```python
from build123d import *

# Parameters (mm, degrees)
BOSS_EXTRUDE1_DEPTH = 1
SKETCH2_W           = 1
SKETCH2_H           = 8.697838108
BOSS_EXTRUDE2_DEPTH = 6
SKETCH3_W           = 3.625858974
SKETCH3_H           = 24.597729298
SKETCH3_R           = 1
BOSS_EXTRUDE3_DEPTH = 1


with BuildPart() as part:
    # Sketch1 → Boss-Extrude1 (new body)
    with BuildSketch(Plane.XY):
        with BuildLine():
            Line((117.275298476, 4.348919054), (20.445206114, 4.348919054))
            ThreePointArc((20.445206114, 4.348919054), (0, 20.902620649), (-20.445206114, 4.348919054))
            Line((-20.445206114, 4.348919054), (-117.275298476, 4.348919054))
            Line((-117.275298476, 4.348919054), (-117.275298476, -4.348919054))
            Line((-117.275298476, -4.348919054), (-20.445206114, -4.348919054))
            ThreePointArc((-20.445206114, -4.348919054), (-16.73157253, -12.528927754), (-9.927442271, -18.394712283))
            Line((-9.927442271, -18.394712283), (-9.927442271, -11.244816137))
            ThreePointArc((-9.927442271, -11.244816137), (-13.314654662, -6.907964333), (-14.909922164, -1.641408252))
            Line((-14.909922164, -1.641408252), (-19.244314933, -1.641408252))
            Line((-19.244314933, -1.641408252), (-19.244314933, 1.641408252))
            Line((-19.244314933, 1.641408252), (-14.909922164, 1.641408252))
            ThreePointArc((-14.909922164, 1.641408252), (0, 15), (14.909922164, 1.641408252))
            Line((14.909922164, 1.641408252), (19.244314933, 1.641408252))
            Line((19.244314933, 1.641408252), (19.244314933, -1.641408252))
            Line((19.244314933, -1.641408252), (14.909922164, -1.641408252))
            ThreePointArc((14.909922164, -1.641408252), (13.314654662, -6.907964333), (9.927442271, -11.244816137))
            Line((9.927442271, -11.244816137), (9.927442271, -18.394712283))
            ThreePointArc((9.927442271, -18.394712283), (16.73157253, -12.528927754), (20.445206114, -4.348919054))
            Line((20.445206114, -4.348919054), (117.275298476, -4.348919054))
            Line((117.275298476, -4.348919054), (117.275298476, 4.348919054))
        make_face()
    extrude(amount=-BOSS_EXTRUDE1_DEPTH)

    # Sketch2 → Boss-Extrude2 (add)
    with BuildSketch(Plane.XY):
        with Locations((-116.775298476, 0)):
            Rectangle(SKETCH2_W, SKETCH2_H)
        with Locations((116.775298476, 0)):
            Rectangle(SKETCH2_W, SKETCH2_H)
    extrude(amount=-BOSS_EXTRUDE2_DEPTH)

    # Sketch3 → Boss-Extrude3 (add)
    # profile 1 of 2: a face of its own
    with BuildSketch(Plane.XY.offset(-6)):
        with Locations((-116.275298476, 0)):
            Rectangle(SKETCH3_W, SKETCH3_H)
        with Locations((-116.275298476, -10)):
            Circle(SKETCH3_R, mode=Mode.SUBTRACT)
        with Locations((-116.275298476, 10)):
            Circle(SKETCH3_R, mode=Mode.SUBTRACT)
    # profile 2 of 2: a face of its own
    with BuildSketch(Plane.XY.offset(-6)):
        with Locations((116.275298476, 0)):
            Rectangle(SKETCH3_W, SKETCH3_H)
        with Locations(Location((116.275298476, 10, 0), (0, 0, 180))):
            Circle(SKETCH3_R, mode=Mode.SUBTRACT)
        with Locations(Location((116.275298476, -10, 0), (0, 0, 180))):
            Circle(SKETCH3_R, mode=Mode.SUBTRACT)
    extrude(amount=BOSS_EXTRUDE3_DEPTH)


solid = part.part
```
The listing builds one solid part. Answer for the finished solid, in the listing's coordinates (mm). A direction names the side the tool comes from. Round coordinates to 2 decimals unless told otherwise and drop trailing zeros. Write each loop counter-clockwise with the first axis right and the second up, starting at its lowest first coordinate (ties: lowest second). Pieces come first, ordered by that corner, then holes. Notation, with made-up numbers: (-39, 70) -> (18, 70) arc R19 ccw to (18, 76) -> close; hole circle Ø3 at (74, 63). An arc over 180 degrees is marked (long way). Answer as a JSON object with one key per item and string values. Group by question number.
Q1. Straight lines are drawn through the part: line 1 along X through (y, z) = (2, -2.5); line 2 along X through (y, z) = (-5.5, -5.6); line 3 along Y through (x, z) = (82, -0.6). For each, find the intervals that lie inside material, in ascending order.
Q2. Section B-B (x = 48) is taken. Write down the section's boundary in (y, z).
Q3. Section A-A (z = -2) is taken. Write down the section's boundary in (x, y).
Q4. Each of these flat-tipped pins is pushed along its axis until it touches: pin 1 Ø1.5 at (x, z) = (-78.5, -3.5) entering from +Y; pin 2 Ø0.8 at (x, z) = (117, -5.5) entering from +Y; pin 3 Ø1.1 at (x, z) = (116.5, -5.5) entering from -Y; pin 4 Ø0.8 at (y, z) = (-0.5, -0.5) entering from +X. Where does it stop, or does it pass through?
Q5. Which of the six approach directions +Z, -Z, +X, -X, +Y, -Y give full straight-line access (tool end or side, diameter ignored) to faces 4 (the face through (-116.275, 0, -3)), 5 (the face through (-117.275, 0, -2)), 6 (the face through (-0.307, 14.997, -0.493))?
Q6. Determine the mould class of faces 1 (the face through (16.655, -12.63, -0.493)), 2 (the face through (116, 0, -6)), 3 (the face through (13.35, -6.84, -0.49)) for opening direction Y: pulls with the +Y half, pulls with the -Y half, needs draft (parallel to the pull), parting line crosses it, or undercut.
Check values:
{
 "1": {"line 1": "-117.28 to -116.28, 116.28 to 117.28", "line 2": "-118.09 to -114.46, 114.46 to 118.09", "line 3": "-4.35 to 4.35"},
 "2": {"outline": "(-4.35, -1) -> (4.35, -1) -> (4.35, 0) -> (-4.35, 0) -> close"},
 "3": {"outline": "(-117.28, -4.35) -> (-116.28, -4.35) -> (-116.28, 4.35) -> (-117.28, 4.35) -> close; (116.28, -4.35) -> (117.28, -4.35) -> (117.28, 4.35) -> (116.28, 4.35) -> close"},
 "4": {"pin 1": "through", "pin 2": "y = 12.3", "pin 3": "y = -12.3", "pin 4": "x = 117.28"},
 "5": {"face 4": "+Y, -Y", "face 5": "+Z, -X, +Y, -Y", "face 6": "+Z, -Z"},
 "6": {"face 1": "pulls with the -Y half", "face 2": "needs draft", "face 3": "undercut"}
}
